Read the model definition and answer for the solid it produces. Units are mm, in the model's axes. Face numbers are marked on the shaded views. A direction names the side the tool comes from. Round coordinates to 2 decimals unless told otherwise and drop trailing zeros. Order: outer loops, then holes, each group sorted by start corner. A loop starts at its lowest first (then second) coordinate and runs counter-clockwise, first axis right, second up.
from build123d import *

# Parameters (mm, degrees)
CUT_EXTRUDE1_DEPTH = 0.75


with BuildPart() as part:
    # Logo3_bib1 → Revolve1 (revolve)
    with BuildSketch(Plane(origin=(0, 0, 0), x_dir=(-1, 0, 0), z_dir=(0, -1, 0))):
        with BuildLine():
            Line((0, -5), (0, 2))
            Line((0, 2), (1.25, 2))
            ThreePointArc((1.25, 2), (1.603553391, 1.853553391), (1.75, 1.5))
            Line((1.75, 1.5), (1.75, 0))
            Line((1.75, 0), (1, 0))
            Line((1, 0), (1, -0.01))
            Line((1, -0.01), (1.013425636, -0.01))
            ThreePointArc((1.013425636, -0.01), (0.993729481, -0.026527036), (1.006585234, -0.048793852))
            Line((1.006585234, -0.048793852), (1, -0.046397023))
            Line((1, -0.046397023), (1, -4.9))
            Line((1, -4.9), (0.9, -5))
            Line((0.9, -5), (0, -5))
        make_face()
    revolve(axis=Axis((0, 0, -10.585154653), (0, 0, 1)))

    # Logo3_bib2 → Cut-Extrude1 (cut)
    with BuildSketch(Plane(origin=(0, 0, -2), x_dir=(1, 0, 0), z_dir=(0, 0, -1))):
        Polygon((0.866025404, 0), (0.433012702, 0.75), (-0.433012702, 0.75), (-0.866025404, 0), (-0.433012702, -0.75), (0.433012702, -0.75), align=None)
    extrude(amount=-CUT_EXTRUDE1_DEPTH, mode=Mode.SUBTRACT)


solid = part.part
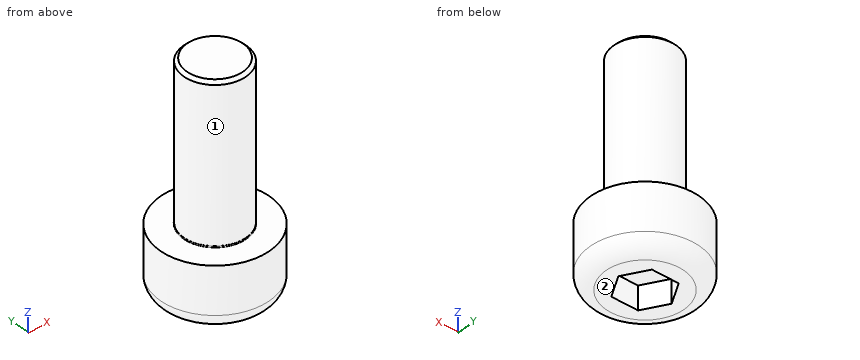
Q1. Straight lines are drawn through the part: probe 1 along Z at (x, y) = (0.1, -0.7); probe 2 along X at (y, z) = (-0.5, 0.25); probe 3 along Z at (x, y) = (0.05, 1.1). For each, find the intervals that lie inside material, in ascending order.
Outcome:
probe 1: z = -1.25 to 5
probe 2: x = -0.87 to 0.87
probe 3: z = -2 to 0
Q2. A cutting plane is placed at B-B, the plane z = 0.75. Give the vertices of the cut face in (x, y).
Outcome:
outline: circle Ø2 at (0, 0)
Q3. For the marked faces 1 and 2, determine the directions among +Z, -Z, +X, -X, +Y, -Y from which every point of the face is accessible in a straight line to the end or side of a thin tool.
Outcome:
face 1: +Z
face 2: -Z, +X, -X, +Y, -Y
Q4. Flat-ended cylindrical pins translate along their axes: pin 1 (1.5 mm diameter, centred on x = 1, z = -0.5, fed in from -Y); pin 2 (1 mm diameter, centred on y = 1, z = 0, fed in from -X). Find the tip coordinate at first contact, or state that the pin passes through.
Outcome:
pin 1: stops at y = -1.73
pin 2: stops at x = -1.68
